Source: CAD feature listing. Evaluate the final solid. Frame: model axes, mm. Give positions to 0.01 mm unless a question says otherwise; leave off trailing zeros. Loops run counter-clockwise (first coordinate to the right, second up) from the corner with the lowest first, then second, coordinate; pieces in that order, holes last. Notation, with made-up numbers: M 66.5,10.5 L 108.5,10.5 A24 cw 108.5,42.5 Z; hole C 79.25,42.5 d5. An arc over 180 degrees is marked long. Answer in a Markdown table with one row per item.
```python
from build123d import *

# Parameters (mm, degrees)
SKETCH_1_R      = 1.55
EXTRUDE_1_DEPTH = 1.5
FILLET_1_R      = 1.5
FILLET_2_R      = 3


with BuildPart() as part:
    # 草图1 → 凸台-拉伸1 (new body)
    with BuildSketch(Plane(origin=(0, 0, 0), x_dir=(1, 0, 0), z_dir=(0, 1, 0))):
        Polygon((27, -4), (27, 4), (11, 4), (4, 11), (4, 27), (-4, 27), (-4, 6), (6, -4), align=None)
        with Locations(Location((15, 0, 0), (0, 0, 270))):
            Circle(SKETCH_1_R, mode=Mode.SUBTRACT)
        with Locations(Location((23, 0, 0), (0, 0, 270))):
            Circle(SKETCH_1_R, mode=Mode.SUBTRACT)
        with Locations(Location((0, 23, 0), (0, 0, 90))):
            Circle(SKETCH_1_R, mode=Mode.SUBTRACT)
        with Locations(Location((0, 15, 0), (0, 0, 90))):
            Circle(SKETCH_1_R, mode=Mode.SUBTRACT)
        with BuildLine():
            Line((2.164213562, 9.164213562), (9.164213562, 2.164213562))
            ThreePointArc((9.164213562, 2.164213562), (9.164213562, -0.664213562), (6.335786438, -0.664213562))
            Line((6.335786438, -0.664213562), (-0.664213562, 6.335786438))
            ThreePointArc((-0.664213562, 6.335786438), (-0.664213562, 9.164213562), (2.164213562, 9.164213562))
        make_face(mode=Mode.SUBTRACT)
    extrude(amount=EXTRUDE_1_DEPTH)

    # 圆角1
    fillet_1_edges = [part.edges().sort_by_distance(p)[0] for p in [
        (-4, 0.75, -27),
        (4, 0.75, -27),
        (27, 0.75, -4),
        (27, 0.75, 4),
    ]]
    fillet(fillet_1_edges, radius=FILLET_1_R)

    # 圆角2
    fillet_2_edges = [part.edges().sort_by_distance(p)[0] for p in [
        (6, 0.75, 4),
        (-4, 0.75, -6),
        (4, 0.75, -11),
        (11, 0.75, -4),
    ]]
    fillet(fillet_2_edges, radius=FILLET_2_R)


solid = part.part
```
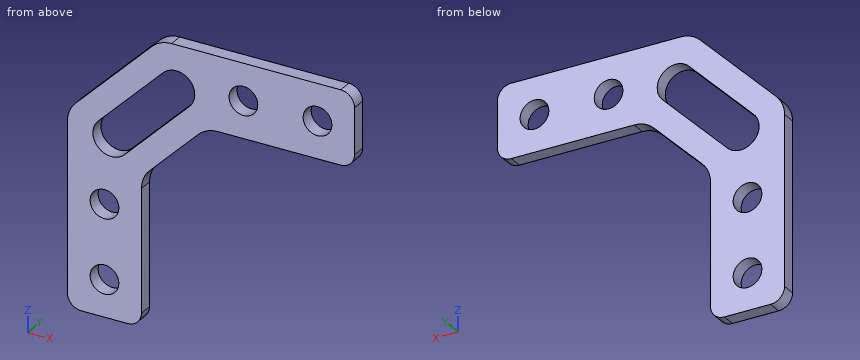
Q1. Section query A-A (z = -15). Output: boundary loops of the cut face in (x, y), plus the area to 3 significant figures.
Values follow:
| item | result |
|---|---|
| outline | M -4,0 L -1.55,0 L -1.55,1.5 L -4,1.5 Z; M 1.55,0 L 4,0 L 4,1.5 L 1.55,1.5 Z |
| area | 7.35 mm^2 |
Q2. Section query B-B (y = 0.25). Output: boundary loops of the cut face in (x, z), plus the area to 3 significant figures.
Values follow:
| item | result |
|---|---|
| outline | M -4,-25.5 A1.5 ccw -2.5,-27 L 2.5,-27 A1.5 ccw 4,-25.5 L 4,-12.24 A3 cw 4.88,-10.12 L 10.12,-4.88 A3 cw 12.24,-4 L 25.5,-4 A1.5 ccw 27,-2.5 L 27,2.5 A1.5 ccw 25.5,4 L 7.24,4 A3 ccw 5.12,3.12 L -3.12,-5.12 A3 ccw -4,-7.24 Z; hole C 0,-23 d3.1; hole C 0,-15 d3.1; hole M -0.66,-6.34 A2 ccw 2.16,-9.16 L 9.16,-2.16 A2 ccw 6.34,0.66 Z; hole C 15,0 d3.1; hole C 23,0 d3.1 |
| area | 322 mm^2 |
Q3. Contact query for flat-ended pins moving along their axis: pin 1 Ø0.8 at (x, y) = (16, 1) entering from -Z; pin 2 Ø0.8 at (y, z) = (0.5, -17.5) entering from +X; pin 3 Ø3 at (x, z) = (0, -15) entering from +Y. Output: stop coordinate, or through.
Values follow:
| item | result |
|---|---|
| pin 1 | z = -4 |
| pin 2 | x = 4 |
| pin 3 | through |
Q4. Section query D-D (z = -0.75). Output: boundary loops of the cut face in (x, y).
Values follow:
| item | result |
|---|---|
| outline | M 1.25,0 L 4.92,0 L 4.92,1.5 L 1.25,1.5 Z; M 9.75,0 L 13.64,0 L 13.64,1.5 L 9.75,1.5 Z; M 16.36,0 L 21.64,0 L 21.64,1.5 L 16.36,1.5 Z; M 24.36,0 L 27,0 L 27,1.5 L 24.36,1.5 Z |
Q5. Ray query, probe 1 along X at (y, z) = (0.5, 0); probe 2 along X at (y, z) = (0.4, -23); probe 3 along Z at (x, y) = (-1, 0.7). Return the intervals inside material, ascending. Write a range as from..to.
Values follow:
| item | result |
|---|---|
| probe 1 | 2..5.67, 9.6..13.45, 16.55..21.45, 24.55..27 |
| probe 2 | -4..-1.55, 1.55..4 |
| probe 3 | -27..-24.18, -21.82..-16.18, -13.82..-8.72, -6.78..-3 |
Q6. Section query C-C (x = 15). Output: boundary loops of the cut face in (y, z).
Values follow:
| item | result |
|---|---|
| outline | M 0,-4 L 1.5,-4 L 1.5,-1.55 L 0,-1.55 Z; M 0,1.55 L 1.5,1.55 L 1.5,4 L 0,4 Z |
